Verification items for the finished model (mm, model axes). A direction names the side the tool comes from. Round coordinates to 2 decimals unless told otherwise and drop trailing zeros. Write each loop counter-clockwise with the first axis right and the second up, starting at its lowest first coordinate (ties: lowest second). Pieces come first, ordered by that corner, then holes. Notation, with made-up numbers: (-39.5, -20) -> (-20.5, -20) arc R19 ccw to (-20.5, -9) -> close; hole circle Ø1 at (-12, 11). An arc over 180 degrees is marked (long way). Answer as a JSON object with one key per item and string values. Group by question number.
(1) Set-up check for faces 4 (the face through (90, 25, 4)), 5 (the face through (75, 17, 0)), 6 (the face through (83.098, 24.994, -0.55)), 7 (the face through (0.21, 40.53, -12.14)), 8 (the face through (-0.21, 40.53, 12.14)): record each of +Z, -Z, +X, -X, +Y, -Y from which the full face is reachable in a straight line by a thin tool's end or side.
(2) Sectioned sample at C-C on y = 31. Count the separate pieces of the cut face and the enclosed holes in it, and give its area (3 significant figures).
(3) Sectioned sample at D-D on x = -1. Record the cut outline in (y, z), and give its area (3 significant figures).
(4) Draft check along Z on faces 1 (the face through (76, 10, 0)), 2 (the face through (-75, 41, 1)), 3 (the face through (-1.05, 19.61, 15.73)). Enter one of: released by +Z, released by -Z, zero draft, split by the parting line, or undercut.
(5) Gauge pin test, flat ends, axial feed: pin 1 Ø1 at (x, z) = (24.5, -24) entering from -Y; pin 2 Ø5 at (y, z) = (22.5, 19.5) entering from +X; pin 3 Ø1.5 at (x, z) = (-56, 13) entering from +Y. Record the tip position at first contact, or that the pin passes through.
(6) Sectioned sample at A-A on x = 45. Record the cut outline in (y, z).
(7) Scan lines: L1, parallel to X at y = 34.5, z = 28.5; L2, parallel to X at y = 55.5, z = 1; L3, parallel to X at y = 46, z = 6.5. Record each from-to range of solid material in increasing order. Write a range as from..to.
(8) Sectioned sample at B-B on z = 0. Record the cut outline in (x, y), and give its area (3 significant figures).
```python
from build123d import *

# Parameters (mm, degrees)
HALF_SPLIT_CUT_DEPTH         = 94
HALF_SPLIT_CUT_DEPTH_BACK    = 80
HALF_SPLIT_CUT_SKETCH_W      = 233.621052632
HALF_SPLIT_CUT_SKETCH_H      = 71.905263158
GRIP_BOSS_DRAFTED_5DEG_DEPTH = 65
GRIP_BOSS_DRAFTED_5DEG_DRAFT = 5
GRIP_BOSS_FILLET_R3_R        = 3
HOOK_END_RECESS_SKETCH_50_R  = 25
HOOK_END_RECESS_50X14_DEPTH  = 14


with BuildPart() as part:
    # Hook Body Profile → Hook Body Revolve (revolve)
    with BuildSketch(Plane.XY, mode=Mode.PRIVATE) as hook_body_revolve_sk:
        with BuildLine():
            Line((-90, 0), (-75, 0))
            Line((-75, 0), (-75, 35))
            Line((-75, 35), (-75, 57.5))
            ThreePointArc((-75, 57.5), (-82.5, 65), (-90, 57.5))
            Line((-90, 57.5), (-90, 0))
        make_face()
        Polygon((-75, 0), (0, 0), (75, 0), (75, 15), (-75, 35), align=None)
        with BuildLine():
            Line((75, 15), (75, 0))
            Line((75, 0), (90, 0))
            Line((90, 0), (90, 27.5))
            ThreePointArc((90, 27.5), (82.5, 35), (75, 27.5))
            Line((75, 27.5), (75, 15))
        make_face()
    revolve(hook_body_revolve_sk.sketch.rotate(Axis((0, 0, 0), (1, 0, 0)), 90), axis=Axis((0, 0, 0), (1, 0, 0)))

    # Half Split Cut Sketch → Half Split Cut (cut, two sides: drawn at the far end of the back side and taken through both)
    with BuildSketch(Plane.XY.offset(-HALF_SPLIT_CUT_DEPTH_BACK)):
        with Locations((-1.705263158, -35.952631579)):
            Rectangle(HALF_SPLIT_CUT_SKETCH_W, HALF_SPLIT_CUT_SKETCH_H)
    extrude(amount=HALF_SPLIT_CUT_DEPTH + HALF_SPLIT_CUT_DEPTH_BACK, mode=Mode.SUBTRACT)


with BuildPart() as grip_boss_drafted_5deg_tool:
    # Grip Boss Sketch 40x20 → Grip Boss Drafted 5deg (with draft: the straight prism first)
    with BuildSketch(Plane(origin=(0, 65, 0), x_dir=(1, 0, 0), z_dir=(0, 1, 0))):
        with BuildLine():
            ThreePointArc((-15, 10), (-18.535533906, 8.535533906), (-20, 5))
            Line((-20, 5), (-20, -5))
            ThreePointArc((-20, -5), (-18.535533906, -8.535533906), (-15, -10))
            Line((-15, -10), (15, -10))
            ThreePointArc((15, -10), (18.535533906, -8.535533906), (20, -5))
            Line((20, -5), (20, 5))
            ThreePointArc((20, 5), (18.535533906, 8.535533906), (15, 10))
            Line((15, 10), (-15, 10))
        make_face()
    extrude(amount=-GRIP_BOSS_DRAFTED_5DEG_DEPTH)
    # Grip Boss Drafted 5deg: the draft: its side faces are tilted about the plane it starts from
    grip_boss_drafted_5deg_sides = [grip_boss_drafted_5deg_tool.faces().sort_by_distance(p)[0] for p in [
        (-18.535533906, 32.5, -8.535533906),
        (-20, 32.5, 0),
        (-18.535533906, 32.5, 8.535533906),
        (0, 32.5, 10),
        (18.535533906, 32.5, 8.535533906),
        (20, 32.5, 0),
        (18.535533906, 32.5, -8.535533906),
        (0, 32.5, -10),
    ]]
    draft(grip_boss_drafted_5deg_sides, Plane(origin=(0, 65, 0), x_dir=(1, 0, 0), z_dir=(0, 1, 0)), GRIP_BOSS_DRAFTED_5DEG_DRAFT)


with BuildPart() as part_1:
    add(part.part)

    # Grip Boss Drafted 5deg: add grip_boss_drafted_5deg_tool
    add(grip_boss_drafted_5deg_tool.part)

    # Grip Boss Fillet R3
    grip_boss_fillet_r3_edges = [part_1.edges().sort_by_distance(p)[0] for p in [
        (18.535533906, 65, -8.535533906),
        (0, 65, -10),
        (-18.535533906, 65, -8.535533906),
        (-20, 65, 0),
        (-18.535533906, 65, 8.535533906),
        (0, 65, 10),
        (18.535533906, 65, 8.535533906),
        (20, 65, 0),
    ]]
    fillet(grip_boss_fillet_r3_edges, radius=GRIP_BOSS_FILLET_R3_R)

    # Hook End Recess Sketch Ø50 → Hook End Recess Ø50x14 (cut)
    with BuildSketch(Plane(origin=(90, 0, 0), x_dir=(0, 0, -1), z_dir=(1, 0, 0))):
        Circle(HOOK_END_RECESS_SKETCH_50_R)
    extrude(amount=-HOOK_END_RECESS_50X14_DEPTH, mode=Mode.SUBTRACT)


solid = part_1.part
```
Computed values:
{
 "1": {"face 4": "+Z, -Z, +X, +Y, -Y", "face 5": "+Y", "face 6": "+X, -Y", "face 7": "-Z, +Y", "face 8": "+Z, +Y"},
 "2": {"separate pieces": "3", "enclosed holes": "0", "area": "3,790 mm2"},
 "3": {"outline": "(0, -25.13) arc R25.13 ccw to (20.97, -13.85) -> (62.26, -10.24) arc R3 ccw to (65, -7.25) -> (65, 7.25) arc R3 ccw to (62.26, 10.24) -> (20.97, 13.85) arc R25.13 ccw to (0, 25.13) -> close", "area": "1,960 mm2"},
 "4": {"face 1": "undercut", "face 2": "zero draft", "face 3": "split by the parting line"},
 "5": {"pin 1": "through", "pin 2": "x = 90", "pin 3": "y = 30.09"},
 "6": {"outline": "(0, -19) arc R19 ccw to (0, 19) -> close"},
 "7": {"L1": "-90..-75", "L2": "-90..-75, -20.83..20.83", "L3": "-90..-75, -21.49..21.49"},
 "8": {"outline": "(-90, 0) -> (76, 0) -> (76, 25) -> (90, 25) -> (90, 27.5) arc R7.5 ccw to (75, 27.5) -> (75, 15) -> (23.78, 21.83) -> (20.24, 62.26) arc R3 ccw to (17.25, 65) -> (-17.25, 65) arc R3 ccw to (-20.24, 62.26) -> (-23.23, 28.1) -> (-75, 35) -> (-75, 57.5) arc R7.5 ccw to (-90, 57.5) -> close", "area": "6,590 mm2"}
}
